For this review, take the finished solid that the model builds, in its own axes (mm). Face numbers are marked on the shaded views. A direction names the side the tool comes from. Round coordinates to 2 decimals unless told otherwise and drop trailing zeros. Write each loop counter-clockwise with the first axis right and the second up, starting at its lowest first coordinate (ties: lowest second). Pieces come first, ordered by that corner, then holes. Notation, with made-up numbers: (-35, -38.5) - (17, -38.5) arc R32 cw to (17, -10.5) - close; hole circle Ø1 at (49.25, 34.25). An arc over 180 degrees is marked (long way). Answer in a Markdown table with one row per item. Add a question column.
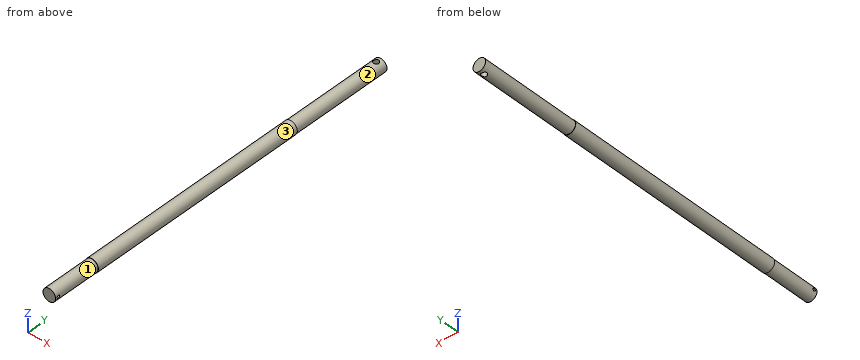
from build123d import *

# Parameters (mm, degrees)
SKETCH1_R               = 12
BOSS_EXTRUDE1_DEPTH     = 90
SKETCH2_R               = 12.5
BOSS_EXTRUDE2_DEPTH     = 420
SKETCH3_R               = 12
BOSS_EXTRUDE3_DEPTH     = 190
CUT_EXTRUDE1_DEPTH      = 701.223178708
CUT_EXTRUDE1_DEPTH_BACK = 701.223178708
SKETCH4_R               = 5.1
CUT_EXTRUDE2_DEPTH      = 701.223178808
CUT_EXTRUDE2_DEPTH_BACK = 701.223178808
SKETCH5_R               = 2.5


with BuildPart() as part:
    # Sketch1 → Boss-Extrude1 (new body)
    with BuildSketch(Plane(origin=(0, 0, 0), x_dir=(1, 0, 0), z_dir=(0, 1, 0))):
        with Locations(Location((0, 0, 0), (0, 0, 90))):
            Circle(SKETCH1_R)
    extrude(amount=BOSS_EXTRUDE1_DEPTH)

    # Sketch2 → Boss-Extrude2 (add)
    with BuildSketch(Plane(origin=(0, 90, 0), x_dir=(1, 0, 0), z_dir=(0, 1, 0))):
        with Locations(Location((0, 0, 0), (0, 0, 270))):
            Circle(SKETCH2_R)
    extrude(amount=BOSS_EXTRUDE2_DEPTH)

    # Sketch3 → Boss-Extrude3 (add)
    with BuildSketch(Plane(origin=(0, 510, 0), x_dir=(1, 0, 0), z_dir=(0, 1, 0))):
        with Locations(Location((0, 0, 0), (0, 0, 90))):
            Circle(SKETCH3_R)
    extrude(amount=BOSS_EXTRUDE3_DEPTH)

    # Sketch4 → Cut-Extrude1 (cut, two sides: drawn at the far end of the back side and taken through both)
    with BuildSketch(Plane.XY.offset(-CUT_EXTRUDE1_DEPTH_BACK)):
        with Locations(Location((0, 690, 0), (0, 0, 90))):
            Circle(SKETCH4_R)
    extrude(amount=CUT_EXTRUDE1_DEPTH + CUT_EXTRUDE1_DEPTH_BACK, mode=Mode.SUBTRACT)

    # Sketch5 → Cut-Extrude2 (cut, two sides: drawn at the far end of the back side and taken through both)
    with BuildSketch(Plane(origin=(0, 0, 0), x_dir=(0, 0, -1), z_dir=(1, 0, 0)).offset(-CUT_EXTRUDE2_DEPTH_BACK)):
        with Locations((0, 6)):
            Circle(SKETCH5_R)
    extrude(amount=CUT_EXTRUDE2_DEPTH + CUT_EXTRUDE2_DEPTH_BACK, mode=Mode.SUBTRACT)


solid = part.part
Q1. Add section B-B on y = 168. State the section outline as (x, z) points.
Q2. To check wall thickness, follow probe 1 along Y at (x, z) = (0.5, 1.25); probe 2 along Z at (x, y) = (0.5, 6); probe 3 along Z at (x, y) = (0.75, 555.5). State the ranges of each line that lie inside material, in increasing order.
Q3. Add section A-A on y = 652.5. State the section outline as (x, z) points.
Q4. Tool access review of the marked faces 1, 2 and 3: name each direction out of +Z, -Z, +X, -X, +Y, -Y from which nothing blocks a thin tool from reaching the whole face with its end or side.
Q5. Insertion check: pin 1 Ø6 at (x, y) = (-5, 71.5) entering from +Z; pin 2 Ø1 at (y, z) = (528, -7) entering from -X; pin 3 Ø1.5 at (x, y) = (-3.5, 222.5) entering from +Z. Each pin has a flat end and moves straight along its axis. Give the tip position at first contact, or say it passes through.
Answer sheet:
| question | item | result |
|---|---|---|
| 1 | outline | circle Ø25 at (0, 0) |
| 2 | probe 1 | y = 0 to 3.83, 8.17 to 684.92, 695.08 to 700 |
| 2 | probe 2 | z = -11.99 to -2.5, 2.5 to 11.99 |
| 2 | probe 3 | z = -11.98 to 11.98 |
| 3 | outline | circle Ø24 at (0, 0) |
| 4 | face 1 | -Y |
| 4 | face 2 | +Y |
| 4 | face 3 | +Y, -Y |
| 5 | pin 1 | stops at z = 11.83 |
| 5 | pin 2 | stops at x = -10.09 |
| 5 | pin 3 | stops at z = 12.19 |
